```python
from build123d import *

# Parameters (mm, degrees)
POCKET_HOUSING_DEPTH                   = 70
SWIVEL_BOSS_DEPTH                      = 25
SWIVEL_BLOCK_DEPTH                     = 15
SWIVEL_PIN_HOLE_SKETCH_R               = 5
SWIVEL_PIN_HOLE_10_DEPTH               = 161.312195419
CLEVIS_START                           = 10
CLEVIS_LUG_DEPTH                       = 10
LUG_HUB_SKETCH_R                       = 20
LUG_HUB_DEPTH                          = 5
LUG_BORE_20_DEPTH                      = 190.076704012
LUG_BORE_20_DEPTH_BACK                 = 190.076704012
LUG_BORE_SKETCH_R                      = 10
PIVOT_BOSS_SKETCH_R                    = 20
PIVOT_BOSS_40_DEPTH                    = 80
PIVOT_COUNTERBORED_HOLE_10_D           = 10
PIVOT_COUNTERBORED_HOLE_10_CBORE_D     = 20
PIVOT_COUNTERBORED_HOLE_10_CBORE_DEPTH = 20
MOUNTING_TAB_DEPTH                     = 15
TAB_COUNTERBORED_HOLE_10_D             = 10
TAB_COUNTERBORED_HOLE_10_CBORE_D       = 20
TAB_COUNTERBORED_HOLE_10_CBORE_DEPTH   = 5


with BuildPart() as part:
    # Pocket Housing Sketch → Pocket Housing (new body)
    with BuildSketch(Plane(origin=(0, 0, 0), x_dir=(1, 0, 0), z_dir=(0, 1, 0))):
        with BuildLine():
            Line((0, 0), (0, 25))
            ThreePointArc((0, 25), (-4.393398282, 35.606601718), (-15, 40))
            Line((-15, 40), (-110, 40))
            ThreePointArc((-110, 40), (-150, 0), (-110, -40))
            Line((-110, -40), (-15, -40))
            ThreePointArc((-15, -40), (-4.393398282, -35.606601718), (0, -25))
            Line((0, -25), (0, 0))
        make_face()
        with BuildLine():
            Line((-15, 30), (-110, 30))
            ThreePointArc((-110, 30), (-140, 0), (-110, -30))
            Line((-110, -30), (-15, -30))
            ThreePointArc((-15, -30), (-11.464466094, -28.535533906), (-10, -25))
            Line((-10, -25), (-10, 0))
            Line((-10, 0), (-10, 25))
            ThreePointArc((-10, 25), (-11.464466094, 28.535533906), (-15, 30))
        make_face(mode=Mode.SUBTRACT)
    extrude(amount=POCKET_HOUSING_DEPTH)

    # Swivel Boss Sketch → Swivel Boss (add)
    with BuildSketch(Plane(origin=(0, 0, 0), x_dir=(1, 0, 0), z_dir=(0, 1, 0))):
        with BuildLine():
            Line((-100, 30), (-100, -30))
            Line((-100, -30), (-110, -30))
            ThreePointArc((-110, -30), (-140, 0), (-110, 30))
            Line((-110, 30), (-100, 30))
        make_face()
    extrude(amount=SWIVEL_BOSS_DEPTH)

    # Swivel Block Sketch → Swivel Block (add)
    with BuildSketch(Plane(origin=(0, 25, 0), x_dir=(1, 0, 0), z_dir=(0, 1, 0))):
        with BuildLine():
            Line((-125, -10), (-138.284271247, -10))
            ThreePointArc((-138.284271247, -10), (-140, 0), (-138.284271247, 10))
            Line((-138.284271247, 10), (-125, 10))
            ThreePointArc((-125, 10), (-115, 0), (-125, -10))
        make_face()
    extrude(amount=SWIVEL_BLOCK_DEPTH)

    # Swivel Pin Hole Sketch → Swivel Pin Hole Ø10 (cut, through all)
    with BuildSketch(Plane(origin=(0, 40, 0), x_dir=(1, 0, 0), z_dir=(0, 1, 0))):
        with Locations(Location((-125, 0, 0), (0, 0, 270))):
            Circle(SWIVEL_PIN_HOLE_SKETCH_R)
    extrude(amount=-SWIVEL_PIN_HOLE_10_DEPTH, mode=Mode.SUBTRACT)

    # Clevis Lug Sketch → Clevis Lug (add)
    with BuildSketch(Plane.XY.offset(CLEVIS_START)):
        with BuildLine():
            Line((0, 70), (34.238039414, 91.857645278))
            ThreePointArc((34.238039414, 91.857645278), (60.501975118, 87.636802105), (59.342535653, 61.061145275))
            Line((59.342535653, 61.061145275), (0, 0))
            Line((0, 0), (0, 70))
        make_face()
    clevis_lug = extrude(amount=CLEVIS_LUG_DEPTH)

    # Lug Hub Sketch → Lug Hub (add)
    with BuildSketch(Plane.XY.offset(20)):
        with Locations(Location((45, 75, 0), (0, 0, 122.554257086))):
            Circle(LUG_HUB_SKETCH_R)
    lug_hub = extrude(amount=LUG_HUB_DEPTH)

    # Clevis Lug Mirror: Clevis Lug, Lug Hub across plane
    add(clevis_lug.mirror(Plane.XY))
    add(lug_hub.mirror(Plane.XY))

    # Lug Bore Sketch → Lug Bore Ø20 (cut, two sides: drawn at the far end of the back side and taken through both)
    with BuildSketch(Plane.XY.offset(25).offset(-LUG_BORE_20_DEPTH_BACK)):
        with Locations(Location((45, 75, 0), (0, 0, 180))):
            Circle(LUG_BORE_SKETCH_R)
    extrude(amount=LUG_BORE_20_DEPTH + LUG_BORE_20_DEPTH_BACK, mode=Mode.SUBTRACT)

    # Pivot Boss Sketch → Pivot Boss Ø40 (add)
    with BuildSketch(Plane.XY.offset(40)):
        with Locations((-65, 35)):
            Circle(PIVOT_BOSS_SKETCH_R)
    extrude(amount=-PIVOT_BOSS_40_DEPTH)

    # Pivot Counterbored Hole Ø10 (through all)
    with Locations(Plane(origin=(-65, 35, 40), x_dir=(1, 0, 0), z_dir=(0, 0, 1))):
        with Locations((0, 0)):
            CounterBoreHole(PIVOT_COUNTERBORED_HOLE_10_D / 2, PIVOT_COUNTERBORED_HOLE_10_CBORE_D / 2, PIVOT_COUNTERBORED_HOLE_10_CBORE_DEPTH)

    # Mounting Tab Sketch → Mounting Tab (add)
    with BuildSketch(Plane(origin=(0, 0, 0), x_dir=(1, 0, 0), z_dir=(0, 1, 0))):
        with BuildLine():
            Line((0, 25), (0, 55))
            ThreePointArc((0, 55), (-8.792955835, 68.655497162), (-24.863013699, 66.301369863))
            Line((-24.863013699, 66.301369863), (-55, 40))
            Line((-55, 40), (-15, 40))
            ThreePointArc((-15, 40), (-4.393398282, 35.606601718), (0, 25))
        make_face()
        with BuildLine():
            Line((0, -25), (0, -55))
            ThreePointArc((0, -55), (-8.792955835, -68.655497162), (-24.863013699, -66.301369863))
            Line((-24.863013699, -66.301369863), (-55, -40))
            Line((-55, -40), (-15, -40))
            ThreePointArc((-15, -40), (-4.393398282, -35.606601718), (0, -25))
        make_face()
    extrude(amount=MOUNTING_TAB_DEPTH)

    # Tab Counterbored Hole Ø10 (through all)
    with Locations(Plane(origin=(-15, 15, 55), x_dir=(0, 0, 1), z_dir=(0, 1, 0))):
        with Locations((0, 0), (-110, 0)):
            CounterBoreHole(TAB_COUNTERBORED_HOLE_10_D / 2, TAB_COUNTERBORED_HOLE_10_CBORE_D / 2, TAB_COUNTERBORED_HOLE_10_CBORE_DEPTH)


solid = part.part
```
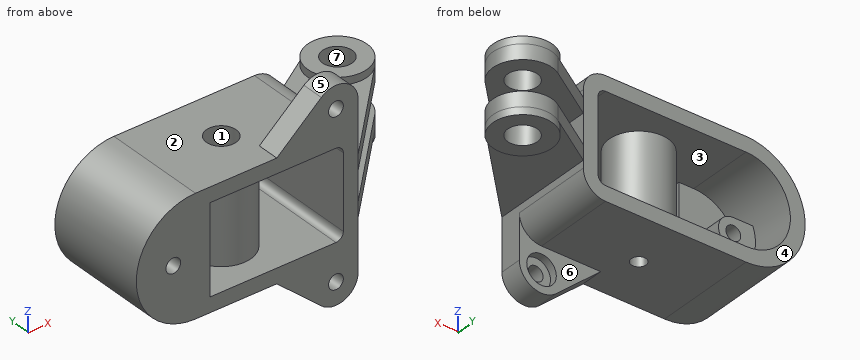
Verification items for the finished model (mm, model axes). Face numbers are marked on the shaded views. A direction names the side the tool comes from. Give positions to 0.01 mm unless a question says otherwise; leave off trailing zeros. Loops run counter-clockwise (first coordinate to the right, second up) from the corner with the lowest first, then second, coordinate; pieces in that order, holes last. Notation, with made-up numbers: M 61,24 L 103,24 A34 ccw 103,61 Z; hole C 85.5,-17.75 d1. An arc over 180 degrees is marked long. One line per question, with ' | ' between items.
Item 1: Section check C-C, the plane y = 75. Record the cut outline in (x, z), plus the area to 3 significant figures.
Completed:
outline: M 7.83,-20 L 25,-20 L 25,-25 L 35,-25 L 35,-10 L 7.83,-10 Z; M 7.83,10 L 35,10 L 35,25 L 25,25 L 25,20 L 7.83,20 Z; M 55,-25 L 65,-25 L 65,-10 L 55,-10 Z; M 55,10 L 65,10 L 65,25 L 55,25 Z | area: 943 mm^2
Item 2: Tool access check on the marked faces 1, 2, 3 and 4. Record the directions out of +Z, -Z, +X, -X, +Y, -Y that give a thin tool (end or side, any length) a straight path to the whole face; none if there is none.
Completed:
face 1: +Z | face 2: +Z, -X, +Y | face 3: none | face 4: +Z, -Z, -X, +Y
Item 3: Section check D-D, the plane x = 44. Record the cut outline in (y, z), plus the area to 3 significant figures.
Completed:
outline: M 45.27,-20 L 55.03,-20 L 55.03,-25 L 65.05,-25 L 65.05,-10 L 45.27,-10 Z; M 45.27,10 L 65.05,10 L 65.05,25 L 55.03,25 L 55.03,20 L 45.27,20 Z; M 84.95,-25 L 94.97,-25 L 94.97,-10 L 84.95,-10 Z; M 84.95,10 L 94.97,10 L 94.97,25 L 84.95,25 Z | area: 797 mm^2
Item 4: Thickness scan on line 1 (Y direction, x = -65, z = 26.25); line 2 (Y direction, x = -65, z = 33); line 3 (X direction, y = 34, z = -26). Record the ranges inside material, lowest first. Write a range as [from, to].
Completed:
line 1: y = [15, 25], [45, 55] | line 2: y = [0, 25], [45, 70] | line 3: x = [-140.4, -124.97], [-84.97, -69.9], [-60.1, -45.03], [-10.1, -0.03]
Item 5: Section check B-B, the plane z = 0. Record the cut outline in (x, y).
Completed:
outline: M -150,0 L -130,0 L -130,40 L -140,40 L -140,70 L -150,70 Z; M -120,0 L -100,0 L -100,25 L -115,25 L -115,40 L -120,40 Z; C -65,35 d40; M -10,0 L 0,0 L 0,70 L -10,70 Z; hole C -65,35 d10
Item 6: Depth check by flat-ended pin: P1, Ø10, axis at x = -1.5, y = 57.5, coming from the +Z side; P2, Ø6, axis at y = 29.5, z = 1, coming from the +X side; P3, Ø10.5, axis at x = -131, y = 31, coming from the -Z side. Enter the tip coordinate at first touch or a pass-through.
Completed:
P1: stops at z = 37.36 | P2: stops at x = 0 | P3: stops at z = -36.77
Item 7: Draft check along X on the marked faces 5, 6 and 7. Enter one of: +X half, -X half, draft (parallel to the pull), parting line (faces both ways), or undercut.
Completed:
face 5: parting line | face 6: draft | face 7: undercut
Item 8: Section check A-A, the plane x = -88. Record the cut outline in (y, z).
Completed:
outline: M 0,-40 L 70,-40 L 70,-30 L 0,-30 Z; M 0,30 L 70,30 L 70,40 L 0,40 Z
